from build123d import *

# Parameters (mm, degrees)
SKETCH_1_W      = 30
SKETCH_1_H      = 61
SKETCH_1_R      = 10
EXTRUDE_1_DEPTH = 2.5
FILLET_1_R      = 5


with BuildPart() as part:
    # 草图1 → 凸台-拉伸1 (new, symmetric)
    with BuildSketch(Plane.XY):
        Rectangle(SKETCH_1_W, SKETCH_1_H)
        with Locations((0, 15.5)):
            Circle(SKETCH_1_R, mode=Mode.SUBTRACT)
    extrude(amount=EXTRUDE_1_DEPTH, both=True)

    # 圆角1
    fillet_1_edges = [part.edges().sort_by_distance(p)[0] for p in [
        (-15, 30.5, 0),
        (15, 30.5, 0),
    ]]
    fillet(fillet_1_edges, radius=FILLET_1_R)


solid = part.part
Here's how the part is built. I have some questions about the finished solid (model axes, mm). Give positions to 0.01 mm unless a question says otherwise; leave off trailing zeros. Write each loop counter-clockwise with the first axis right and the second up, starting at its lowest first coordinate (ties: lowest second). Pieces come first, ordered by that corner, then holes. Notation, with made-up numbers: (83, 84.5) -> (128, 84.5) arc R16 cw to (128, 103.5) -> close; hole circle Ø1 at (37.25, 28). An arc over 180 degrees is marked (long way). Use one line per item in the form item = value. Start each with the question number.
1. Thinking about a two-plate mould opening in Y: for faces 1 (the face through (-1.302, 25.415, -0.035)), 2 (the face through (-15, -3, 0)), 3 (the face through (13.57, 29, -0.04)), which applies, +Y half, -Y half, draft (parallel to the pull), parting line (faces both ways), or undercut?
2. Imagine slicing it at A-A on x = 0. List the corners of the cut face in (y, z) for me, plus the area to 3 significant figures.
3. Imagine slicing it at B-B on y = 15.5. List the corners of the cut face in (x, z) for me.
4. If I drill on L1, parallel to Y at x = 0, z = 0.1; L2, parallel to Y at x = 6, z = -0.75; L3, parallel to X at y = 13, z = 0.25, over which ranges is the centre line in solid material (lowest first)?
5. Will this pin go through, and if not, where does the flat tip stop? pin 1 Ø16 at (x, y) = (0, 15.5) entering from -Z.
6. Imagine slicing it at C-C on z = -1.85. List the corners of the cut face in (x, y) for me.
Entries:
q1.face_1 = undercut
q1.face_2 = draft
q1.face_3 = +Y half
q2.outline = (-30.5, -2.5) -> (5.5, -2.5) -> (5.5, 2.5) -> (-30.5, 2.5) -> close; (25.5, -2.5) -> (30.5, -2.5) -> (30.5, 2.5) -> (25.5, 2.5) -> close
q2.area = 205 mm²
q3.outline = (-15, -2.5) -> (-10, -2.5) -> (-10, 2.5) -> (-15, 2.5) -> close; (10, -2.5) -> (15, -2.5) -> (15, 2.5) -> (10, 2.5) -> close
q4.L1 = -30.5 to 5.5, 25.5 to 30.5
q4.L2 = -30.5 to 7.5, 23.5 to 30.5
q4.L3 = -15 to -9.68, 9.68 to 15
q5.pin_1 = through
q6.outline = (-15, -30.5) -> (15, -30.5) -> (15, 25.5) arc R5 ccw to (10, 30.5) -> (-10, 30.5) arc R5 ccw to (-15, 25.5) -> close; hole circle Ø20 at (0, 15.5)
